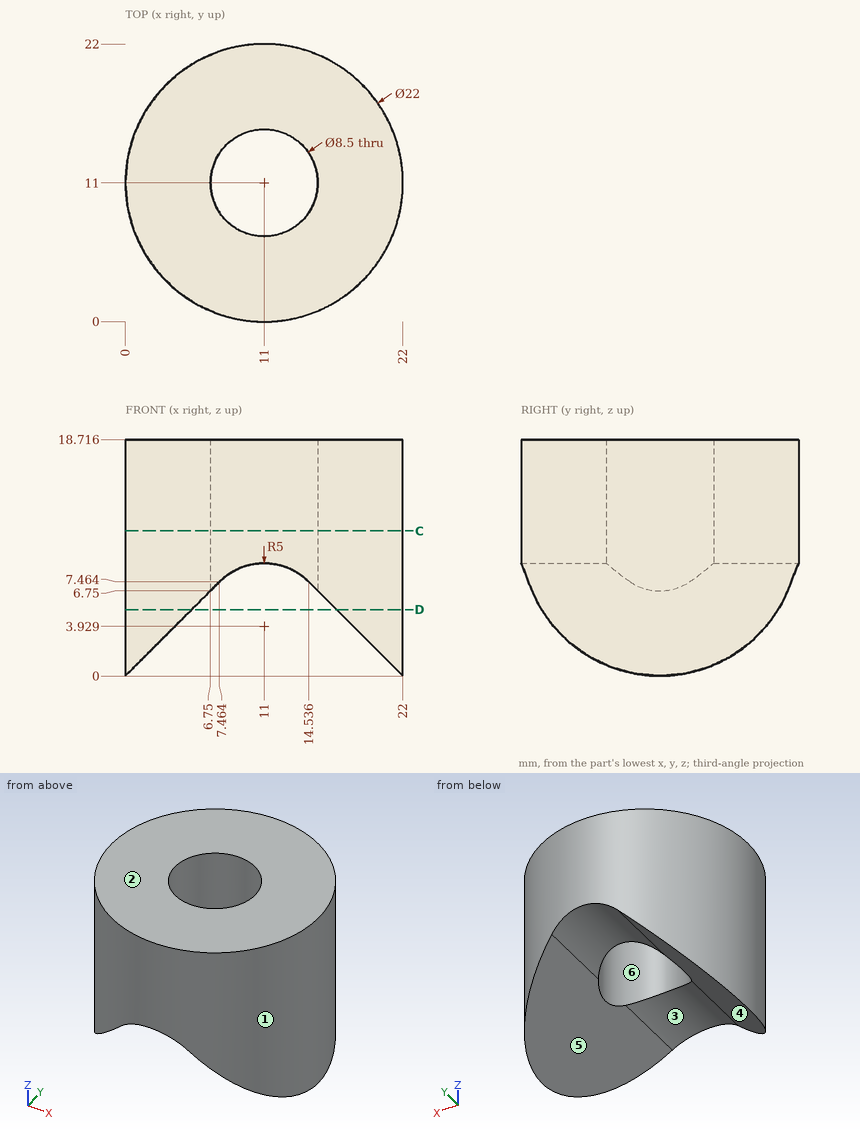
Geometry: see drawing. Coordinates: mm, zero at the bounding-box minimum. A direction names the side the tool comes from. Give positions to 0.01 mm unless a question says otherwise; leave off trailing zeros. Order: outer loops, then holes, each group sorted by start corner. A loop starts at its lowest first (then second) coordinate and runs counter-clockwise, first axis right, second up. Notation, with made-up numbers: (-3, -24.5) - (27, -24.5) arc R22 cw to (27, -3.5) - close; hole circle Ø1 at (7, 35). An arc over 180 degrees is marked (long way). One line per item, written item: value.
1. Cut plane C-C, the plane z = 11.5. Output: boundary loops of the cut face in (x, y), and give its area (3 significant figures).
Determined:
outline: circle Ø22 at (11, 11); hole circle Ø8.5 at (11, 11)
area: 323 mm2
2. Pin query (flat end, axial travel): pin 1 Ø10 at (x, y) = (3.5, 17.5) entering from -Z; pin 2 Ø1 at (y, z) = (12, 6) entering from +X; pin 3 Ø5 at (y, z) = (6, 8) entering from +X. Return the tip coordinate at first contact, or that it passes through.
Determined:
pin 1: z = 0.32
pin 2: x = 21.99
pin 3: x = 21.71
3. Draft query along X for the marked faces 1, 2, 3 and 4. Return one class per face: released by +X, released by -X, zero draft, split by the parting line, or undercut.
Determined:
face 1: split by the parting line
face 2: zero draft
face 3: undercut
face 4: undercut
4. Line query: probe 1 along Y at (x, z) = (11, 9.5); probe 2 along X at (y, z) = (14.25, 15); probe 3 along X at (y, z) = (10.5, 15.5). Output: solid intervals per line, ascending.
Determined:
probe 1: 0 to 6.75, 15.25 to 22
probe 2: 0.49 to 8.26, 13.74 to 21.51
probe 3: 0.01 to 6.78, 15.22 to 21.99
5. Reachability of the marked faces 5 and 6 from +Z, -Z, +X, -X, +Y, -Y: full face, straight path, thin tool, end or side. Return the list, or none.
Determined:
face 5: -Z, +Y, -Y
face 6: +Z, -Z
6. Cut plane D-D, the plane z = 5.25. Output: boundary loops of the cut face in (x, y).
Determined:
outline: (5.25, 1.62) - (5.25, 20.38) arc R11 ccw to start; (16.75, 1.62) arc R11 ccw to (16.75, 20.38) - close
